Work out the finished part from the listing and answer in its coordinate system (mm). A direction names the side the tool comes from. Round coordinates to 2 decimals unless told otherwise and drop trailing zeros. Write each loop counter-clockwise with the first axis right and the second up, starting at its lowest first coordinate (ties: lowest second). Pieces come first, ordered by that corner, then holes. Notation, with made-up numbers: (10, 82.25) - (22, 82.25) arc R12 ccw to (22, 102.25) - close; hole circle Ø9 at (43, -27). An arc over 180 degrees is marked (long way). Answer as a JSON object with one key per item and string values.
```python
from build123d import *

# Parameters (mm, degrees)
SKETCH_1_W               = 20
SKETCH_1_H               = 20
SKETCH_1_R               = 1.94442565
EXTRUDE_1_DEPTH          = 101
CUT_EXTRUDE_1_DEPTH      = 203.494444368
PATTERN_CIRCULAR_1_COUNT = 4


with BuildPart() as part:
    # 草图1 → 凸台-拉伸1 (new, symmetric)
    with BuildSketch(Plane.XY):
        Rectangle(SKETCH_1_W, SKETCH_1_H)
        Circle(SKETCH_1_R, mode=Mode.SUBTRACT)
    extrude(amount=EXTRUDE_1_DEPTH, both=True)

    # 草图2 → 切除-拉伸1 (cut, symmetric)
    with BuildSketch(Plane.XY.offset(101)):
        Polygon((-32.933615203, 60.643738676), (-3.694439046, 10), (-2.5, 7.931170886), (2.5, 7.931170886), (3.694439046, 10), (32.933615203, 60.643738676), (32.933615203, 177.600443305), (-32.933615203, 177.600443305), align=None)
    cut_extrude_1 = extrude(amount=CUT_EXTRUDE_1_DEPTH, both=True, mode=Mode.SUBTRACT)

    # 阵列(圆周)1: 切除-拉伸1 ×4 about axis
    pattern_circular_1_axis = Axis((0, 0, 101), (0, 0, -1))
    for i in range(1, PATTERN_CIRCULAR_1_COUNT):
        add(cut_extrude_1.rotate(pattern_circular_1_axis, i * 360 / PATTERN_CIRCULAR_1_COUNT), mode=Mode.SUBTRACT)


solid = part.part
```
Item 1: Determine the mould class of faces 5 (the cylindrical face through (-0.42, -1.9, -1.41)), 6 (the flat face through (-7.931, 0, 1)), 7 (the flat face through (-10, -7, 1)), 8 (the flat face through (-7, 10, 1)) for opening direction Y: pulls with the +Y half, pulls with the -Y half, needs draft (parallel to the pull), parting line crosses it, or undercut.
Results found:
{"face 5": "undercut", "face 6": "undercut", "face 7": "needs draft", "face 8": "pulls with the +Y half"}
Item 2: For faces 1 (the flat face through (0, 7.931, 1)), 2 (the flat face through (0, -7.931, 1)), 3 (the flat face through (10, 7, 1)), 4 (the flat face through (7.931, 0, 1)), determine the directions among +Z, -Z, +X, -X, +Y, -Y from which every point of the face is accessible in a straight line to the end or side of a thin tool.
Results found:
{"face 1": "+Z, -Z, +Y", "face 2": "+Z, -Z, -Y", "face 3": "+Z, -Z, +X, +Y, -Y", "face 4": "+Z, -Z, +X"}
Item 3: Each of these flat-tipped pins is pushed along its axis until it touches: P1, Ø10, axis at y = -1, z = -22.5, coming from the +X side; P2, Ø2.5, axis at y = -0.5, z = 25, coming from the -X side; P3, Ø5.5, axis at x = 0, z = -20, coming from the -Y side; P4, Ø4, axis at y = 1, z = 1.5, coming from the +X side. Where does it stop, or does it pass through?
Results found:
{"P1": "x = 10", "P2": "x = -7.93", "P3": "y = -8.36", "P4": "x = 8.8"}
Item 4: A cutting plane is placed at C-C (z = -59). Write down the section's boundary in (x, y).
Results found:
{"outline": "(-10, -10) - (-3.69, -10) - (-2.5, -7.93) - (2.5, -7.93) - (3.69, -10) - (10, -10) - (10, -3.69) - (7.93, -2.5) - (7.93, 2.5) - (10, 3.69) - (10, 10) - (3.69, 10) - (2.5, 7.93) - (-2.5, 7.93) - (-3.69, 10) - (-10, 10) - (-10, 3.69) - (-7.93, 2.5) - (-7.93, -2.5) - (-10, -3.69) - close; hole circle Ø3.89 at (0, 0)"}
Item 5: Consider line 1 along Y through (x, z) = (0, 41); line 2 along Y through (x, z) = (8, 44); line 3 along X through (y, z) = (1.75, 62). Determine where each line is inside the solid, lowest interval first.
Results found:
{"line 1": "-7.93 to -1.94, 1.94 to 7.93", "line 2": "-10 to -2.54, 2.54 to 10", "line 3": "-7.93 to -0.85, 0.85 to 7.93"}
Item 6: A cutting plane is placed at A-A (x = 0). Write down the section's boundary in (y, z).
Results found:
{"outline": "(-7.93, -101) - (-1.94, -101) - (-1.94, 101) - (-7.93, 101) - close; (1.94, -101) - (7.93, -101) - (7.93, 101) - (1.94, 101) - close"}
